```python
from build123d import *

# Parameters (mm, degrees)
BOSS_EXTRUDE1_DEPTH = 220
SHELL1_T            = -2
CUT_EXTRUDE1_DEPTH  = 321.212491043
SKETCH3_R           = 2.5
CUT_EXTRUDE2_DEPTH  = 394.612153142
SKETCH4_W           = 20
SKETCH4_H           = 30
CUT_EXTRUDE3_DEPTH  = 357.766015962
FILLET1_R           = 5
SKETCH5_W           = 50
SKETCH5_H           = 20
CUT_EXTRUDE4_DEPTH  = 376.254580252
FILLET2_R           = 5


with BuildPart() as part:
    # Sketch1 → Boss-Extrude1 (new body)
    with BuildSketch(Plane.XY):
        Polygon((-164.523614444, 0), (-116.335763439, -116.335763439), (0, -164.523614444), (116.335763439, -116.335763439), (164.523614444, 0), (116.335763439, 116.335763439), (0, 164.523614444), (-116.335763439, 116.335763439), align=None)
    extrude(amount=BOSS_EXTRUDE1_DEPTH)

    # Shell1
    shell1_openings = [part.faces().sort_by_distance(p)[0] for p in [
        (0, 0, 220),
        (0, 0, 0),
    ]]
    offset(amount=SHELL1_T, openings=shell1_openings, kind=Kind.INTERSECTION)

    # Sketch2 → Cut-Extrude1 (cut, through all)
    with BuildSketch(Plane.XY.offset(220)):
        Polygon((75.61693775, 182.555436661), (-82.042454152, -198.068005503), (95.714298716, -271.697263345), (253.373690618, 108.92617882), align=None)
    extrude(amount=-CUT_EXTRUDE1_DEPTH, mode=Mode.SUBTRACT)

    # Sketch3 → Cut-Extrude2 (cut, through all)
    with BuildSketch(Plane(origin=(-58.167881719, -140.429688942, 0), x_dir=(0.9238795325112961, -0.3826834323650676, 0), z_dir=(-0.3826834323650675, -0.923879532511296, 0))):
        with Locations((-12, 200)):
            Circle(SKETCH3_R)
        with Locations((-12, 140)):
            Circle(SKETCH3_R)
        with Locations((-12, 80)):
            Circle(SKETCH3_R)
    extrude(amount=-CUT_EXTRUDE2_DEPTH, mode=Mode.SUBTRACT)

    # Sketch4 → Cut-Extrude3 (cut, through all)
    with BuildSketch(Plane(origin=(-140.429688942, 58.167881719, 0), x_dir=(0, 0, 1), z_dir=(-0.9238795325112957, 0.3826834323650681, 0))):
        with Locations((10, -37.960461481)):
            Rectangle(SKETCH4_W, SKETCH4_H)
    extrude(amount=-CUT_EXTRUDE3_DEPTH, mode=Mode.SUBTRACT)

    # Fillet1
    fillet1_edges = [part.edges().sort_by_distance(p)[0] for p in [
        (-148.292397617, 36.572497868, 20),
        (-159.772900588, 8.856111893, 20),
    ]]
    fillet(fillet1_edges, radius=FILLET1_R)

    # Sketch5 → Cut-Extrude4 (cut, through all)
    with BuildSketch(Plane(origin=(-58.167881719, 140.429688942, 0), x_dir=(0.9238795325112777, 0.3826834323651116, 0), z_dir=(-0.38268343236511165, 0.9238795325112779, 0))):
        with Locations((0.039538519, -10)):
            Rectangle(SKETCH5_W, SKETCH5_H)
    extrude(amount=-CUT_EXTRUDE4_DEPTH, mode=Mode.SUBTRACT)

    # Fillet2
    fillet2_edges = [part.edges().sort_by_distance(p)[0] for p in [
        (-34.651681146, 149.088025955, 20),
        (-80.845657771, 129.953854336, 20),
    ]]
    fillet(fillet2_edges, radius=FILLET2_R)


solid = part.part
```
The listing builds one solid part. Answer for the finished solid, in the listing's coordinates (mm). A direction names the side the tool comes from. Give positions to 0.01 mm unless a question says otherwise; leave off trailing zeros. Order: outer loops, then holes, each group sorted by start corner. A loop starts at its lowest first (then second) coordinate and runs counter-clockwise, first axis right, second up. Notation, with made-up numbers: (13.25, -33.75) -> (69.25, -33.75) arc R13 ccw to (69.25, -24.75) -> close; hole circle Ø2 at (-8, 29.5). An arc over 180 degrees is marked (long way). Answer as a JSON object with one key per item and string values. Group by question number.
Item 1: The part is cut by section C-C on y = 120. Write down the section's boundary in (x, z), and give its area (3 significant figures).
Item 2: The part is cut by section B-B on x = -124.5. Write down the section's boundary in (y, z), and give its area (3 significant figures).
Item 3: The part is cut by section A-A on z = 119. Write down the section's boundary in (x, y), and give its area (3 significant figures).
Item 4: Determine the mould class of faces 4 (the flat face through (-154, 23, 20)), 5 (the flat face through (-56.599, 138.915, 108.46)), 6 (the flat face through (-140.77, -57.35, 108.46)) for opening direction X: pulls with the +X half, pulls with the -X half, needs draft (parallel to the pull), parting line crosses it, or undercut.
Item 5: A tool of negligible diameter and unlimited length cuts with its end or side. For faces 1 (the flat face through (-138.249, 58.206, 108.46)), 2 (the flat face through (29.49, 152.31, 108.46)), 3 (the flat face through (29.103, 150.304, 108.46)), from which of +Z, -Z, +X, -X, +Y, -Y can it reach the whole face along a straight path? Write none if from no direction.
Item 6: Flat-ended cylindrical pins translate along their axes: pin 1 (4 mm diameter, centred on x = -97, z = 114, fed in from +Y); pin 2 (13.5 mm diameter, centred on x = -56.5, y = 143, fed in from -Z); pin 3 (1.5 mm diameter, centred on x = -28, z = 116.5, fed in from -Y). Find the tip coordinate at first contact, or state that the pin passes through.
Item 7: Consider L1, parallel to Y at x = -147.5, z = 135; L2, parallel to Y at x = -145, z = 196; L3, parallel to Y at x = 17, z = 208. Determine where each line is inside the solid, lowest interval first. Write a range as from..to.
Item 8: The part is cut by section D-D on x = -15.5. Write down the section's boundary in (y, z), and give its area (3 significant figures).
Result set:
{
 "1": {"outline": "(-107.49, 0) -> (-102.26, 0) -> (-102.26, 220) -> (-107.49, 220) -> close", "area": "1,150 mm²"},
 "2": {"outline": "(-96.63, 0) -> (-91.4, 0) -> (-91.4, 220) -> (-96.63, 220) -> close; (91.4, 0) -> (96.63, 0) -> (96.63, 220) -> (91.4, 220) -> close", "area": "2,300 mm²"},
 "3": {"outline": "(-164.52, 0) -> (-116.34, -116.34) -> (-58.17, -140.43) -> (-57.4, -138.58) -> (-114.81, -114.81) -> (-162.36, 0) -> (-114.81, 114.81) -> (0, 162.36) -> (57.4, 138.58) -> (58.17, 140.43) -> (0, 164.52) -> (-116.34, 116.34) -> close", "area": "1,000 mm²"},
 "4": {"face 4": "needs draft", "face 5": "undercut", "face 6": "pulls with the -X half"},
 "5": {"face 1": "+Z, -Z, +X", "face 2": "+Z, -Z, +X, +Y", "face 3": "+Z, -Z, -Y"},
 "6": {"pin 1": "y = 125.17", "pin 2": "z = 20", "pin 3": "y = 150.45"},
 "7": {"L1": "-41.1..-35.87, 35.87..41.1", "L2": "-47.13..-41.91, 41.91..47.13", "L3": "155.32..157.48"},
 "8": {"outline": "(155.94, 0) -> (158.1, 0) -> (158.1, 220) -> (155.94, 220) -> close", "area": "476 mm²"}
}
